Source: CAD feature listing. Evaluate the final solid. Frame: model axes, mm. Face numbers are marked on the shaded views. A direction names the side the tool comes from. Give positions to 0.01 mm unless a question says otherwise; leave off trailing zeros. Order: outer loops, then holes, each group sorted by start corner. A loop starts at its lowest first (then second) coordinate and runs counter-clockwise, first axis right, second up. Notation, with made-up numbers: M 28,-13.75 L 74,-13.75 A33 cw 74,25.25 Z; hole C 23.25,89.25 d5. An arc over 180 degrees is marked long. Answer in a Markdown table with one row per item. Add a question column.
(1) Section query C-C, the plane y = 41. Return loops of the section in (x, z).
(2) Set-up query: the marked faces 5, 6, 7, 8 and 9. Return all of +Z, -Z, +X, -X, +Y, -Y with unobstructed straight access to the full face (end or side cutting, diameter ignored); none if empty.
(3) Material intervals for line 1 along Z through (x, y) = (50, 8); line 2 along Z through (x, y) = (33, 50); line 3 along Z through (x, y) = (122.5, 12.5), sorted ascending.
(4) Section query D-D, the plane z = 26. Return loops of the section in (x, y).
(5) Mould query, pull axis Y, two halves, no side actions, for the marked faces 1, 2, 3 and 4. Classes: pulls with the +Y half, pulls with the -Y half, needs draft (parallel to the pull), parting line crosses it, or undercut.
(6) Pin query (flat end, axial travel): P1, Ø13, axis at x = 92, y = 77, coming from the +Z side; P2, Ø4, axis at y = 63.5, z = 33, coming from the -X side; P3, Ø5, axis at x = 82, y = 51, coming from the +Z side. Return the tip coordinate at first contact, or that it passes through.
(7) Section query A-A, the plane z = 42. Return loops of the section in (x, y).
(8) Section query B-B, the plane x = 50. Return loops of the section in (y, z).
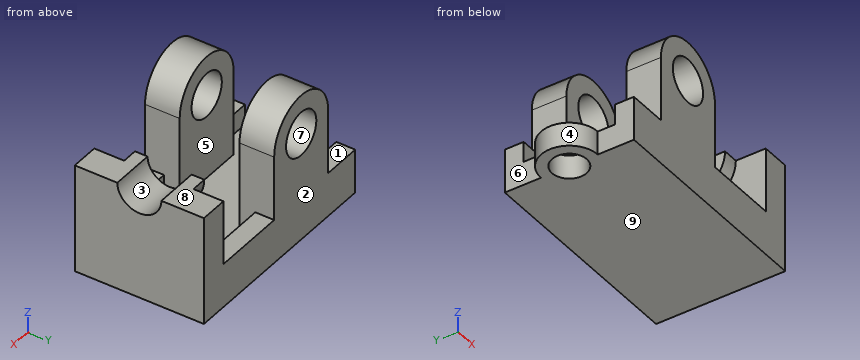
from build123d import *

# Parameters (mm, degrees)
BASE_PLATE_SKETCH_W         = 140
BASE_PLATE_SKETCH_H         = 82
BASE_PLATE_DEPTH            = 15
BACK_WALL_SKETCH_W          = 54
BACK_WALL_SKETCH_H          = 82
BACK_WALL_DEPTH             = 18
REAR_HALF_BOSS_DEPTH        = 10
REAR_HALF_ROUND_CUT_DEPTH   = 28
LOWER_LUG_DEPTH             = 22
SPACER_BLOCK_1_SKETCH_W     = 47
SPACER_BLOCK_1_SKETCH_H     = 13
SPACER_BLOCK_1_DEPTH        = 12
SPACER_BLOCK_2_SKETCH_W     = 25
SPACER_BLOCK_2_SKETCH_H     = 13
SPACER_BLOCK_2_DEPTH        = 12
SPACER_BLOCK_3_SKETCH_W     = 47
SPACER_BLOCK_3_SKETCH_H     = 13
SPACER_BLOCK_3_DEPTH        = 12
UPPER_START                 = -22
UPPER_LUG_DEPTH             = 22
SPACER_BLOCK_4_SKETCH_W     = 25
SPACER_BLOCK_4_SKETCH_H     = 13
SPACER_BLOCK_4_DEPTH        = 12
SIDE_HALF_BOSS_DEPTH        = 15
SIDE_BORE_SKETCH_R          = 11
SIDE_BORE_22_DEPTH          = 15
UPPER_PIN_HOLE_SKETCH_R     = 14
UPPER_LUG_PIN_HOLE_28_DEPTH = 22
LOWER_START                 = -22
LOWER_PIN_HOLE_SKETCH_R     = 14
LOWER_LUG_PIN_HOLE_28_DEPTH = 22


with BuildPart() as part:
    # Base Plate Sketch → Base Plate (new body)
    with BuildSketch(Plane.XY):
        with Locations((70, 41)):
            Rectangle(BASE_PLATE_SKETCH_W, BASE_PLATE_SKETCH_H)
    extrude(amount=BASE_PLATE_DEPTH)

    # Back Wall Sketch → Back Wall (add)
    with BuildSketch(Plane(origin=(140, 0, 0), x_dir=(0, 0, -1), z_dir=(1, 0, 0))):
        with Locations((-42, 41)):
            Rectangle(BACK_WALL_SKETCH_W, BACK_WALL_SKETCH_H)
    extrude(amount=-BACK_WALL_DEPTH)

    # Rear Half Boss Sketch → Rear Half Boss (add)
    with BuildSketch(Plane.ZY.offset(-122)):
        with BuildLine():
            Line((69, 63), (69, 19))
            ThreePointArc((69, 19), (47, 41), (69, 63))
        make_face()
    extrude(amount=REAR_HALF_BOSS_DEPTH)

    # Rear Half-Round Cut Sketch → Rear Half-Round Cut (cut)
    with BuildSketch(Plane.ZY.offset(-112)):
        with BuildLine():
            Line((69, 55), (69, 27))
            ThreePointArc((69, 27), (55, 41), (69, 55))
        make_face()
    extrude(amount=-REAR_HALF_ROUND_CUT_DEPTH, mode=Mode.SUBTRACT)

    # Lower Lug Sketch → Lower Lug (add)
    with BuildSketch(Plane.XZ):
        with BuildLine():
            Line((75, 69), (75, 15))
            Line((75, 15), (25, 15))
            Line((25, 15), (25, 69))
            ThreePointArc((25, 69), (50, 94), (75, 69))
        make_face()
    extrude(amount=-LOWER_LUG_DEPTH)

    # Spacer Block 1 Sketch → Spacer Block 1 (add)
    with BuildSketch(Plane.XZ):
        with Locations((98.5, 21.5)):
            Rectangle(SPACER_BLOCK_1_SKETCH_W, SPACER_BLOCK_1_SKETCH_H)
    extrude(amount=-SPACER_BLOCK_1_DEPTH)

    # Spacer Block 2 Sketch → Spacer Block 2 (add)
    with BuildSketch(Plane.XZ):
        with Locations((12.5, 21.5)):
            Rectangle(SPACER_BLOCK_2_SKETCH_W, SPACER_BLOCK_2_SKETCH_H)
    extrude(amount=-SPACER_BLOCK_2_DEPTH)

    # Spacer Block 3 Sketch → Spacer Block 3 (add)
    with BuildSketch(Plane(origin=(0, 82, 0), x_dir=(1, 0, 0), z_dir=(0, 1, 0))):
        with Locations((98.5, -21.5)):
            Rectangle(SPACER_BLOCK_3_SKETCH_W, SPACER_BLOCK_3_SKETCH_H)
    extrude(amount=-SPACER_BLOCK_3_DEPTH)

    # Upper Lug Sketch → Upper Lug (add)
    with BuildSketch(Plane(origin=(0, 82, 0), x_dir=(1, 0, 0), z_dir=(0, 1, 0)).offset(UPPER_START)):
        with BuildLine():
            Line((25, -15), (75, -15))
            Line((75, -15), (75, -69))
            ThreePointArc((75, -69), (50, -94), (25, -69))
            Line((25, -69), (25, -15))
        make_face()
    extrude(amount=UPPER_LUG_DEPTH)

    # Spacer Block 4 Sketch → Spacer Block 4 (add)
    with BuildSketch(Plane(origin=(0, 82, 0), x_dir=(1, 0, 0), z_dir=(0, 1, 0))):
        with Locations((12.5, -21.5)):
            Rectangle(SPACER_BLOCK_4_SKETCH_W, SPACER_BLOCK_4_SKETCH_H)
    extrude(amount=-SPACER_BLOCK_4_DEPTH)

    # Side Half Boss Sketch → Side Half Boss (add)
    with BuildSketch(Plane.XY.offset(15)):
        with BuildLine():
            Line((0, 59), (0, 23))
            ThreePointArc((0, 23), (-18, 41), (0, 59))
        make_face()
    extrude(amount=-SIDE_HALF_BOSS_DEPTH)

    # Side Bore Sketch → Side Bore Ø22 (cut)
    with BuildSketch(Plane.XY.offset(15)):
        with Locations((0, 41)):
            Circle(SIDE_BORE_SKETCH_R)
    extrude(amount=-SIDE_BORE_22_DEPTH, mode=Mode.SUBTRACT)

    # Upper Pin Hole Sketch → Upper Lug Pin Hole Ø28 (cut)
    with BuildSketch(Plane(origin=(0, 82, 0), x_dir=(1, 0, 0), z_dir=(0, 1, 0))):
        with Locations(Location((50, -69, 0), (0, 0, 270))):
            Circle(UPPER_PIN_HOLE_SKETCH_R)
    extrude(amount=-UPPER_LUG_PIN_HOLE_28_DEPTH, mode=Mode.SUBTRACT)

    # Lower Pin Hole Sketch → Lower Lug Pin Hole Ø28 (cut)
    with BuildSketch(Plane.XZ.offset(LOWER_START)):
        with Locations(Location((50, 69, 0), (0, 0, 90))):
            Circle(LOWER_PIN_HOLE_SKETCH_R)
    extrude(amount=LOWER_LUG_PIN_HOLE_28_DEPTH, mode=Mode.SUBTRACT)


solid = part.part
Values follow:
| question | item | result |
|---|---|---|
| 1 | outline | M -18,0 L -11,0 L -11,15 L -18,15 Z; M 11,0 L 140,0 L 140,55 L 112,55 L 112,47 L 122,47 L 122,15 L 11,15 Z |
| 2 | face 5 | +Z, -X |
| 2 | face 6 | +Z, -Z, -X, +Y |
| 2 | face 7 | +Y, -Y |
| 2 | face 8 | +Z, +X, +Y, -Y |
| 2 | face 9 | -Z, +X, -X, +Y, -Y |
| 3 | line 1 | z = 0 to 55, 83 to 94 |
| 3 | line 2 | z = 0 to 15 |
| 3 | line 3 | z = 0 to 69 |
| 4 | outline | M 0,0 L 140,0 L 140,82 L 0,82 L 0,70 L 25,70 L 25,60 L 75,60 L 75,70 L 122,70 L 122,12 L 75,12 L 75,22 L 25,22 L 25,12 L 0,12 Z |
| 5 | face 1 | needs draft |
| 5 | face 2 | pulls with the +Y half |
| 5 | face 3 | undercut |
| 5 | face 4 | parting line crosses it |
| 6 | P1 | stops at z = 28 |
| 6 | P2 | stops at x = 25 |
| 6 | P3 | stops at z = 15 |
| 7 | outline | M 25,0 L 75,0 L 75,22 L 25,22 Z; M 25,60 L 75,60 L 75,82 L 25,82 Z; M 122,0 L 140,0 L 140,82 L 122,82 Z |
| 8 | outline | M 0,0 L 82,0 L 82,55 L 60,55 L 60,15 L 22,15 L 22,55 L 0,55 Z; M 0,83 L 22,83 L 22,94 L 0,94 Z; M 60,83 L 82,83 L 82,94 L 60,94 Z |
